from build123d import *

# Parameters (mm, degrees)
SKETCH_1_R          = 58
EXTRUDE_1_DEPTH     = 2.4
SKETCH_2_R          = 53
EXTRUDE_2_DEPTH     = 17.4
CHAMFER_1_SIZE      = 2.5
SKETCH_3_R          = 20.5
EXTRUDE_3_DEPTH     = 13.5
SKETCH_4_R          = 18.5
CUT_EXTRUDE_1_DEPTH = 1.1
SKETCH_5_R          = 2.5
CUT_EXTRUDE_2_DEPTH = 320
SKETCH_6_R          = 50.5
CUT_EXTRUDE_3_DEPTH = 16.5
CUT_EXTRUDE_START   = -13
CUT_EXTRUDE_5_DEPTH = 13
EXTRUDE_4_DEPTH     = 2.5
SKETCH_9_W          = 11.6
SKETCH_9_H          = 21.886068862
CUT_EXTRUDE_6_DEPTH = 13.5
EXTRUDE_5_DEPTH     = 39.5
EXTRUDE_START       = -14.047642545
EXTRUDE_6_DEPTH     = 14.047642545
CUT_EXTRUDE_7_REACH = 90.118
SKETCH_10_R         = 9.6


with BuildPart() as part:
    # 草图1 → 凸台-拉伸1 (new body)
    with BuildSketch(Plane.XY):
        Circle(SKETCH_1_R)
    extrude(amount=EXTRUDE_1_DEPTH)

    # 草图2 → 凸台-拉伸2 (add)
    with BuildSketch(Plane.XY.offset(2.4)):
        Circle(SKETCH_2_R)
    extrude(amount=EXTRUDE_2_DEPTH)

    # 倒角1
    chamfer_1_edges = [part.edges().sort_by_distance(p)[0] for p in [
        (-53, 0, 19.8),
    ]]
    chamfer(chamfer_1_edges, length=CHAMFER_1_SIZE)

    # 草图3 → 凸台-拉伸3 (add)
    with BuildSketch(Plane.XY.offset(19.8)):
        Circle(SKETCH_3_R)
    extrude(amount=EXTRUDE_3_DEPTH)

    # 草图4 → 切除-拉伸1 (cut)
    with BuildSketch(Plane.XY.offset(33.3)):
        Circle(SKETCH_4_R)
    extrude(amount=-CUT_EXTRUDE_1_DEPTH, mode=Mode.SUBTRACT)

    # 草图5 → 切除-拉伸2 (cut)
    with BuildSketch(Plane.XY.offset(32.2)):
        with Locations((0, -15.4)):
            Circle(SKETCH_5_R)
        with Locations((-13.336791218, 7.7)):
            Circle(SKETCH_5_R)
        with Locations((13.336791218, 7.7)):
            Circle(SKETCH_5_R)
    extrude(amount=-CUT_EXTRUDE_2_DEPTH, mode=Mode.SUBTRACT)

    # 草图6 → 切除-拉伸3 (cut)
    with BuildSketch(Plane(origin=(0, 0, 0), x_dir=(-1, 0, 0), z_dir=(0, 0, -1))):
        Circle(SKETCH_6_R)
    extrude(amount=-CUT_EXTRUDE_3_DEPTH, mode=Mode.SUBTRACT)

    # 草图7 → 切除-拉伸5 (cut)
    with BuildSketch(Plane(origin=(0, 0, 16.5), x_dir=(-1, 0, 0), z_dir=(0, 0, -1)).offset(CUT_EXTRUDE_START)):
        with BuildLine():
            Line((-11.708521868, 0.986415561), (-17.925222851, 4.575629546))
            ThreePointArc((-17.925222851, 4.575629546), (-16.02146997, -9.25), (-5, -17.811513131))
            Line((-5, -17.811513131), (-5, -10.633085159))
            ThreePointArc((-5, -10.633085159), (-10.175798494, -5.875), (-11.708521868, 0.986415561))
        make_face()
        with BuildLine():
            Line((5, -10.633085159), (5, -17.811513131))
            ThreePointArc((5, -17.811513131), (16.02146997, -9.25), (17.925222851, 4.575629546))
            Line((17.925222851, 4.575629546), (11.708521868, 0.986415561))
            ThreePointArc((11.708521868, 0.986415561), (10.175798494, -5.875), (5, -10.633085159))
        make_face()
        with BuildLine():
            Line((-7, 9.814954576), (-12.925222851, 13.235883584))
            ThreePointArc((-12.925222851, 13.235883584), (-10.150568751, 15.466607709), (-7, 17.12454379))
            Line((-7, 17.12454379), (-7, 9.814954576))
        make_face()
        with BuildLine():
            Line((7, 9.814954576), (12.925222851, 13.235883584))
            ThreePointArc((12.925222851, 13.235883584), (10.150568751, 15.466607709), (7, 17.12454379))
            Line((7, 17.12454379), (7, 9.814954576))
        make_face()
    extrude(amount=CUT_EXTRUDE_5_DEPTH, mode=Mode.SUBTRACT)

    # 草图8 → 凸台-拉伸4 (add)
    with BuildSketch(Plane.XY.offset(19.8)):
        with BuildLine():
            Line((-6, 27.810115066), (6, 27.810115066))
            ThreePointArc((6, 27.810115066), (0, -28.45), (-6, 27.810115066))
        make_face()
        with BuildLine():
            Line((-6, 25.452357455), (6, 25.452357455))
            ThreePointArc((6, 25.452357455), (0, -26.15), (-6, 25.452357455))
        make_face(mode=Mode.SUBTRACT)
    extrude(amount=EXTRUDE_4_DEPTH)

    # 草图9 → 切除-拉伸6 (cut)
    with BuildSketch(Plane.XY.offset(33.3)):
        with Locations((0, 10.943034431)):
            Rectangle(SKETCH_9_W, SKETCH_9_H)
    extrude(amount=-CUT_EXTRUDE_6_DEPTH, mode=Mode.SUBTRACT)

    # 草图11 → 凸台-拉伸5 (add)
    with BuildSketch(Plane(origin=(0, 0, 0), x_dir=(1, 0, 0), z_dir=(0, 1, 0))):
        with BuildLine():
            Line((-3.75, -19.8), (3.75, -19.8))
            Line((3.75, -19.8), (3.75, -23.8))
            ThreePointArc((3.75, -23.8), (0, -21.8), (-3.75, -23.8))
            Line((-3.75, -23.8), (-3.75, -19.8))
        make_face()
    extrude(amount=EXTRUDE_5_DEPTH)

    # 草图12 → 凸台-拉伸6 (add)
    with BuildSketch(Plane(origin=(0, 39.5, 0), x_dir=(1, 0, 0), z_dir=(0, 1, 0)).offset(EXTRUDE_START)):
        with BuildLine():
            Line((-3.75, -23.8), (-3.75, -25.8))
            Line((-3.75, -25.8), (-2.5, -25.8))
            ThreePointArc((-2.5, -25.8), (0, -23.3), (2.5, -25.8))
            Line((2.5, -25.8), (3.75, -25.8))
            Line((3.75, -25.8), (3.75, -23.8))
            ThreePointArc((3.75, -23.8), (0, -21.8), (-3.75, -23.8))
        make_face()
    extrude(amount=EXTRUDE_6_DEPTH)

    # 草图10 → 切除-拉伸7 (cut, up to next)
    with BuildSketch(Plane.XY.offset(32.2), mode=Mode.PRIVATE) as cut_extrude_7_sk1:
        with Locations(Location((0, 0, 0), (0, 0, 52.831100344))):
            Circle(SKETCH_10_R)
    cut_extrude_7_tool1 = extrude(cut_extrude_7_sk1.sketch, amount=-CUT_EXTRUDE_7_REACH, mode=Mode.PRIVATE) & part.part
    add(cut_extrude_7_tool1.solids().sort_by_distance((0, 0, 32.2))[0], mode=Mode.SUBTRACT)


solid = part.part
Can you work these out from the model? Positions are in its coordinate system, mm. A direction names the side the tool comes from. Round coordinates to 2 decimals unless told otherwise and drop trailing zeros. Write each loop counter-clockwise with the first axis right and the second up, starting at its lowest first coordinate (ties: lowest second). Pieces come first, ordered by that corner, then holes. Notation, with made-up numbers: M 22.5,-5 L 60.5,-5 A24 cw 60.5,14 Z; hole C 22.25,72 d3. An arc over 180 degrees is marked long. Use a Markdown table: item, result.
Item 1: Which directions (+Z, -Z, +X, -X, +Y, -Y) give clear straight access to the entire face, cutting with the end or side of a thin tool? Please do faces 5 (the face through (-5.8, 14, 27)), 6 (the face through (-9.92, 11.5, 23.09)), 7 (the face through (-0.1, 32.4, 23.3)).
Found:
| item | result |
|---|---|
| face 5 | +Z |
| face 6 | -Z |
| face 7 | +Z, +Y |
Item 2: If I drill on line 1 along Y through (x, z) = (0, 20.3); line 2 along X through (y, z) = (0, 21); line 3 along Y through (x, z) = (0, 32), over which ranges is the centre line in solid material (lowest first)? Write a range as [from, to].
Found:
| item | result |
|---|---|
| line 1 | y = [-28.45, -26.15], [-20.5, -17.9], [-12.9, -9.6], [9.6, 39.5] |
| line 2 | x = [-28.45, -26.15], [-20.5, -18.5], [-11.75, -9.6], [9.6, 11.75], [18.5, 20.5], [26.15, 28.45] |
| line 3 | y = [-20.5, -17.9], [-12.9, -9.6] |
Item 3: I want a section at B-B (z = 12). List the corners of the cut face in (x, y) for me, and give its area (3 significant figures).
Found:
| item | result |
|---|---|
| outline | C 0,0 d106; hole C 0,0 d101 |
| area | 813 mm2 |
Item 4: For pin 1 Ø10 at (x, y) = (-22.5, 16.5) entering from -Z; pin 2 Ø2 at (y, z) = (-16, 20.5) entering from -X; pin 3 Ø9.5 at (y, z) = (14, 27.5) entering from -X; pin 4 Ø10 at (x, z) = (35, 28.5) entering from +Y, each with a flat end and sliding along its axis, tell me the tip position at first contact or that it passes through.
Found:
| item | result |
|---|---|
| pin 1 | stops at z = 16.5 |
| pin 2 | stops at x = -48.26 |
| pin 3 | stops at x = -18.29 |
| pin 4 | passes through |
Item 5: I want a section at A-A (x = 0). State how many separate pieces and enclosed holes the cut face has, and give its area (3 significant figures).
Found:
| item | result |
|---|---|
| separate pieces | 3 |
| enclosed holes | 0 |
| area | 532 mm2 |
Item 6: We'd pull the mould along X, two halves only. Please class faces 1 (the face through (12, -6, 29.5)), 2 (the face through (-17, 48, 0)), 3 (the face through (10.95, -49.3, 8.13)), 4 (the face through (1.166, -28.426, 21.032)): released by +X, released by -X, zero draft, split by the parting line, or undercut.
Found:
| item | result |
|---|---|
| face 1 | undercut |
| face 2 | zero draft |
| face 3 | undercut |
| face 4 | split by the parting line |
